```python
from build123d import *

# Parameters (mm, degrees)
F_40_X_40_X_4_1_DEPTH = 110


with BuildPart() as part:
    # Sketch12 → 方形管 40 X 40 X 4(1) (new body)
    with BuildSketch(Plane(origin=(0, 0, 0), x_dir=(0, 0, -1), z_dir=(1, 0, 0))):
        with BuildLine():
            Line((-12, -20), (12, -20))
            ThreePointArc((12, -20), (17.656854249, -17.656854249), (20, -12))
            Line((20, -12), (20, 12))
            ThreePointArc((20, 12), (17.656854249, 17.656854249), (12, 20))
            Line((12, 20), (-12, 20))
            ThreePointArc((-12, 20), (-17.656854249, 17.656854249), (-20, 12))
            Line((-20, 12), (-20, -12))
            ThreePointArc((-20, -12), (-17.656854249, -17.656854249), (-12, -20))
        make_face()
        with BuildLine():
            Line((-12, -16), (12, -16))
            ThreePointArc((12, -16), (14.828427125, -14.828427125), (16, -12))
            Line((16, -12), (16, 12))
            ThreePointArc((16, 12), (14.828427125, 14.828427125), (12, 16))
            Line((12, 16), (-12, 16))
            ThreePointArc((-12, 16), (-14.828427125, 14.828427125), (-16, 12))
            Line((-16, 12), (-16, -12))
            ThreePointArc((-16, -12), (-14.828427125, -14.828427125), (-12, -16))
        make_face(mode=Mode.SUBTRACT)
    extrude(amount=F_40_X_40_X_4_1_DEPTH)


solid = part.part
```
Can you work these out from the model? Positions are in its coordinate system, mm. A direction names the side the tool comes from. Round coordinates to 2 decimals unless told otherwise and drop trailing zeros. Loops run counter-clockwise (first coordinate to the right, second up) from the corner with the lowest first, then second, coordinate; pieces in that order, holes last. Notation, with made-up numbers: M 79,9.5 L 123,9.5 A18 ccw 123,38.5 Z; hole C 41,75 d4. An arc over 180 degrees is marked long. Answer as a JSON object with one key per item and string values. Group by question number.
Q1. Please list where these lines run through material, in increasing order: L1, parallel to Y at x = 24, z = 2; L2, parallel to Y at x = 28, z = -15.5.
Q2. We'd pull the mould along Z, two halves only. Please class faces 3 (the flat face through (54, 0, -20)), 4 (the flat face through (110, 0.1, 16.4)), 5 (the cylindrical face through (54.23, -14.859, -14.797)), 6 (the flat face through (54, -16, 0)): +Z half, -Z half, draft (parallel to the pull), parting line (faces both ways), or undercut.
Q3. Will this pin go through, and if not, where does the flat tip stop? pin 1 (1.5 mm diameter, centred on x = 67.5, y = -16, fed in from -Z).
Q4. Imagine slicing it at B-B, the plane z = 2.5. Please give me the cut outline in (x, y).
Q5. On a 3-axis mill with a long thin cutter (end or side, diameter ignored), from which of +Z, -Z, +X, -X, +Y, -Y can I reach the whole of each face in a straight line? I mean faces 1 (the flat face through (54, 20, 0)), 2 (the cylindrical face through (54.23, 14.859, 14.797)). Say none if no direction works.
Q6. Imagine slicing it at D-D, the plane z = -17. Please give me the cut outline in (x, y) (3 decimals), then the cut area to 3 significant figures.
Q7. Imagine slicing it at A-A, the plane x = 15. Please give me the cut outline in (y, z).
Findings:
{
 "1": {"L1": "y = -20 to -16, 16 to 20", "L2": "y = -19.19 to -13.94, 13.94 to 19.19"},
 "2": {"face 3": "-Z half", "face 4": "draft", "face 5": "undercut", "face 6": "undercut"},
 "3": {"pin 1": "stops at z = -19.31"},
 "4": {"outline": "M 0,-20 L 110,-20 L 110,-16 L 0,-16 Z; M 0,16 L 110,16 L 110,20 L 0,20 Z"},
 "5": {"face 1": "+Z, -Z, +X, -X, +Y", "face 2": "+X, -X"},
 "6": {"outline": "M 0,-18.245 L 110,-18.245 L 110,18.245 L 0,18.245 Z", "area": "4,010 mm2"},
 "7": {"outline": "M -20,-12 A8 ccw -12,-20 L 12,-20 A8 ccw 20,-12 L 20,12 A8 ccw 12,20 L -12,20 A8 ccw -20,12 Z; hole M -16,-12 A4 ccw -12,-16 L 12,-16 A4 ccw 16,-12 L 16,12 A4 ccw 12,16 L -12,16 A4 ccw -16,12 Z"}
}
